Geometry check sheet. Reference: drawing and pictorial views, mm from the part's lowest x, y, z. A direction names the side the tool comes from. Round coordinates to 2 decimals unless told otherwise and drop trailing zeros. Write each loop counter-clockwise with the first axis right and the second up, starting at its lowest first coordinate (ties: lowest second). Pieces come first, ordered by that corner, then holes. Notation, with made-up numbers: M 21,34.25 L 79,34.25 A25 ccw 79,54.25 Z; hole C -29.5,22 d7. An arc over 180 degrees is marked long. Use a Markdown table: item, result. Add a question column.
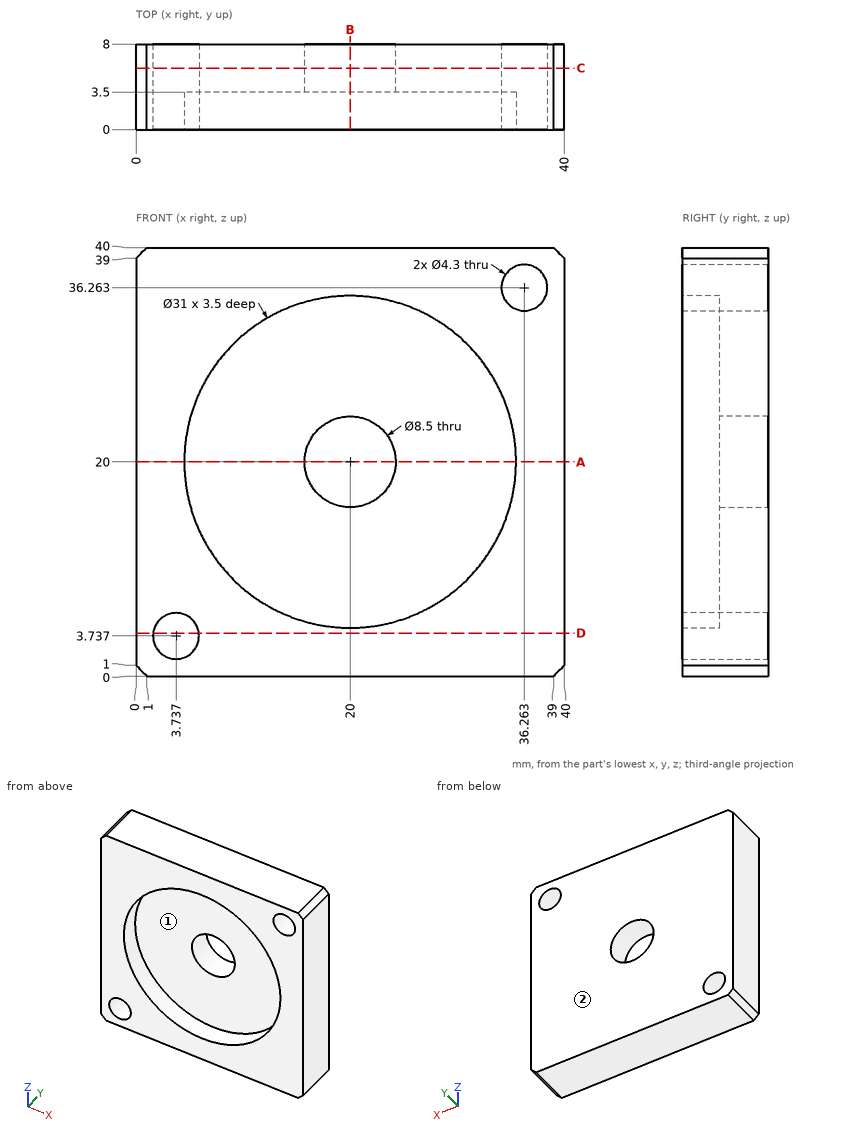
1. Depth check by flat-ended pin: pin 1 Ø15.5 at (x, z) = (23.5, 17) entering from -Y; pin 2 Ø3 at (x, y) = (18, 7) entering from -Z. Enter the tip coordinate at first touch or a pass-through.
2. Cross-section at C-C on y = 5.75. Enter the section's corners in (x, z).
3. Access from +Z, -Z, +X, -X, +Y, -Y to the whole of each face (thin tool, end or side, straight path). Record for the marked faces 1 and 2.
4. Cross-section at B-B on x = 20. Enter the section's corners in (y, z).
5. Scan lines: line 1 along X through (y, z) = (1.8, 20); line 2 along X through (y, z) = (6.35, 20); line 3 along Z through (x, y) = (12, 2) (1 decimal). Record each from-to range of solid material in increasing order. Write a range as from..to.
6. Cross-section at A-A on z = 20. Enter the section's corners in (x, y).
7. Cross-section at D-D on z = 4. Enter the section's corners in (x, y).
Answer:
| question | item | result |
|---|---|---|
| 1 | pin 1 | stops at y = 3.5 |
| 1 | pin 2 | stops at z = 0 |
| 2 | outline | M 0,1 L 1,0 L 39,0 L 40,1 L 40,39 L 39,40 L 1,40 L 0,39 Z; hole C 3.74,3.74 d4.3; hole C 20,20 d8.5; hole C 36.26,36.26 d4.3 |
| 3 | face 1 | -Y |
| 3 | face 2 | +Z, -Z, +X, -X, +Y |
| 4 | outline | M 0,0 L 8,0 L 8,15.75 L 3.5,15.75 L 3.5,4.5 L 0,4.5 Z; M 0,35.5 L 3.5,35.5 L 3.5,24.25 L 8,24.25 L 8,40 L 0,40 Z |
| 5 | line 1 | x = 0..4.5, 35.5..40 |
| 5 | line 2 | x = 0..15.75, 24.25..40 |
| 5 | line 3 | z = 0..6.7, 33.3..40 |
| 6 | outline | M 0,0 L 4.5,0 L 4.5,3.5 L 15.75,3.5 L 15.75,8 L 0,8 Z; M 24.25,3.5 L 35.5,3.5 L 35.5,0 L 40,0 L 40,8 L 24.25,8 Z |
| 7 | outline | M 0,0 L 1.6,0 L 1.6,8 L 0,8 Z; M 5.87,0 L 40,0 L 40,8 L 5.87,8 Z |
